```python
from build123d import *

# Parameters (mm, degrees)
CUT_EXTRUDE1_DEPTH = 5.06


with BuildPart() as part:
    # Sketch1 → Revolve1 (revolve)
    with BuildSketch(Plane.XY):
        with BuildLine():
            Line((0, 4), (-14.870210074, 4))
            ThreePointArc((-14.870210074, 4), (-15.026502525, 4.031798059), (-15.157945994, 4.122136652))
            Line((-15.157945994, 4.122136652), (-19.829816323, 8.96))
            Line((-19.829816323, 8.96), (-20, 8.96))
            Line((-20, 8.96), (-20, 0))
            Line((-20, 0), (0, 0))
            Line((0, 0), (0, 4))
        make_face()
    revolve(axis=Axis((0, 0, 0), (-1, 0, 0)))

    # Sketch2 → Cut-Extrude1 (cut)
    with BuildSketch(Plane.ZY.offset(20)):
        Polygon((0, 2.886751346), (-2.5, 1.443375673), (-2.5, -1.443375673), (0, -2.886751346), (2.5, -1.443375673), (2.5, 1.443375673), align=None)
    extrude(amount=-CUT_EXTRUDE1_DEPTH, mode=Mode.SUBTRACT)

    # Sketch6 → Revolve2 (revolve)
    with BuildSketch(Plane.XY, mode=Mode.PRIVATE) as revolve2_sk:
        Polygon((-17, 2.886751346), (-15.333333333, 0), (-14.22, 0), (-14.22, 2.886751346), align=None)
    revolve(revolve2_sk.sketch.rotate(Axis((-20, 0, 0), (1, 0, 0)), 90), axis=Axis((-20, 0, 0), (1, 0, 0)))

    # Sketch7 → Cut-Revolve2 (revolve, cut)
    with BuildSketch(Plane.XY):
        Polygon((-20, 2.886751346), (-20, 0), (-19.208, 0), align=None)
    revolve(axis=Axis((-20, 0, 0), (1, 0, 0)), mode=Mode.SUBTRACT)

    # Sketch4 → Cut-Revolve1 (revolve, cut)
    with BuildSketch(Plane.XY):
        Polygon((-0.625, 4), (0, 2.917468245), (0.625, 4), align=None)
    revolve(axis=Axis((-0.625, 0, 0), (1, 0, 0)), mode=Mode.SUBTRACT)


solid = part.part
```
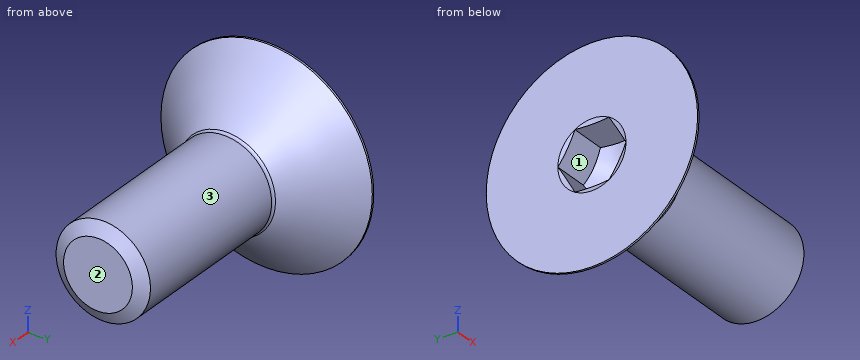
Can you work these out from the model? Positions are in its coordinate system, mm. Face numbers are marked on the shaded views. A direction names the side the tool comes from. Coordinates: 2 decimals unless noted, no trailing zeros. Loops run counter-clockwise (first coordinate to the right, second up) from the corner with the lowest first, then second, coordinate; pieces in that order, holes last. Notation, with made-up numbers: (38, -30) - (97, -30) arc R31 ccw to (97, 2) - close; hole circle Ø10 at (73, -32.5). An arc over 180 degrees is marked (long way). Use a Markdown table: item, result.
Item 1: If I drill on probe 1 along Z at (x, y) = (-3.25, 1); probe 2 along Z at (x, y) = (-18.5, -4); probe 3 along X at (y, z) = (7.5, 0.5), over which ranges is the centre line in solid material (lowest first)? Write a range as from..to.
Numbers:
| item | result |
|---|---|
| probe 1 | z = -3.87..3.87 |
| probe 2 | z = -6.44..6.44 |
| probe 3 | x = -20..-18.44 |
Item 2: For the marked faces 1, 2 and 3, which set-ups out of +Z, -Z, +X, -X, +Y, -Y let a thin tool reach every point of the face, with its end or its side?
Numbers:
| item | result |
|---|---|
| face 1 | -X |
| face 2 | +Z, -Z, +X, +Y, -Y |
| face 3 | +X |
Item 3: I want a section at A-A on x = -8.75. Please give me the cut outline in (y, z), and give its area (3 significant figures).
Numbers:
| item | result |
|---|---|
| outline | circle Ø8 at (0, 0) |
| area | 50.3 mm2 |
Item 4: Will these pins go through, and if not, where does the flat tip stop? pin 1 (1.5 mm diameter, centred on y = 5.5, z = -3, fed in from +X); pin 2 (3 mm diameter, centred on x = -18, y = -0.5, fed in from +Z); pin 3 (3 mm diameter, centred on y = 1, z = 7, fed in from +X).
Numbers:
| item | result |
|---|---|
| pin 1 | stops at x = -16.5 |
| pin 2 | stops at z = 8.61 |
| pin 3 | stops at x = -16.56 |
